from build123d import *

# Parameters (mm, degrees)
SKETCH_1_W                   = 8
SKETCH_1_H                   = 20
EXTRUDE_1_DEPTH              = 10
HOLE_WIZARD_M3_1_D           = 3.4
HOLE_WIZARD_M3_1_CBORE_D     = 6
HOLE_WIZARD_M3_1_CBORE_DEPTH = 6


with BuildPart() as part:
    # 草图1 → 凸台-拉伸1 (new body)
    with BuildSketch(Plane.XY):
        Rectangle(SKETCH_1_W, SKETCH_1_H)
    extrude(amount=EXTRUDE_1_DEPTH)

    # M3 六角圆柱头螺钉的柱形沉头孔1 (through all)
    with Locations(Plane(origin=(4, 0, 0), x_dir=(0, 0, -1), z_dir=(1, 0, 0))):
        with Locations((-5, 5.5), (-5, -5.5)):
            CounterBoreHole(HOLE_WIZARD_M3_1_D / 2, HOLE_WIZARD_M3_1_CBORE_D / 2, HOLE_WIZARD_M3_1_CBORE_DEPTH)

    # 草图4 → 切除-旋转1 (revolve, cut)
    with BuildSketch(Plane(origin=(0, 0, 0), x_dir=(1, 0, 0), z_dir=(0, 1, 0))):
        Polygon((11.5, 1.5), (0.5, 1.5), (1.200682375, -13.581690109), (11.5, -13.581690109), align=None)
    revolve(axis=Axis((11.5, 0, 13.581690109), (0, 0, -1)), mode=Mode.SUBTRACT)


solid = part.part
Work out the finished part from the listing and answer in its coordinate system (mm). A direction names the side the tool comes from. Give positions to 0.01 mm unless a question says otherwise; leave off trailing zeros. Write each loop counter-clockwise with the first axis right and the second up, starting at its lowest first coordinate (ties: lowest second). Pieces come first, ordered by that corner, then holes. Notation, with made-up numbers: (64.5, -4) - (83.5, -4) arc R24 cw to (83.5, 35) - close; hole circle Ø4 at (32.25, 17.5). An arc over 180 degrees is marked (long way). One line per item, written item: value. Start each with the question number.
1. For a pull along Y with two mould halves and no side action, classify faces 3 (the flat face through (4, 9, 5)), 4 (the flat face through (0, 10, 5)), 5 (the flat face through (-2, -7.5, 5)) as +Y half, -Y half, draft (parallel to the pull), parting line (faces both ways), or undercut.
2. Consider probe 1 along Y at (x, z) = (-0.5, 5); probe 2 along Y at (x, z) = (1.5, 5); probe 3 along Y at (x, z) = (-1, 3.75). Determine where each line is inside the solid, lowest interval first.
3. Find section D-D (x = -2.75). Write down the section's boundary in (y, z), then the cut area to 3 significant figures.
4. Find section A-A (x = -1). Write down the section's boundary in (y, z), then the cut area to 3 significant figures.
5. Find section B-B (z = 5). Write down the section's boundary in (x, y).
6. For faces 1 (the flat face through (4, -9, 5)), 2 (the cylindrical face through (0.375, 8.474, 5.391)), determine the directions among +Z, -Z, +X, -X, +Y, -Y from which every point of the face is accessible in a straight line to the end or side of a thin tool.
7. Find section C-C (z = 7). Write down the section's boundary in (x, y).
8. Given pin 1 (1.8 mm diameter, centred on y = -6, z = 6, fed in from +X); pin 2 (2.5 mm diameter, centred on y = 5.5, z = 5, fed in from -X), each flat-ended and moving along its own axis, determine where each tip first touches the part or whether it passes through.
Geometry results:
1. face 3: draft
1. face 4: +Y half
1. face 5: undercut
2. probe 1: -10 to -8.5, -2.5 to 2.5, 8.5 to 10
2. probe 2: -10 to -8.5, 8.5 to 10
2. probe 3: -10 to -8.23, -2.77 to 2.77, 8.23 to 10
3. outline: (-10, 0) - (10, 0) - (10, 10) - (-10, 10) - close; hole circle Ø3.4 at (-5.5, 5); hole circle Ø3.4 at (5.5, 5)
3. area: 182 mm2
4. outline: (-10, 0) - (10, 0) - (10, 10) - (-10, 10) - close; hole circle Ø6 at (-5.5, 5); hole circle Ø6 at (5.5, 5)
4. area: 143 mm2
5. outline: (-4, -10) - (4, -10) - (4, -8.5) - (-2, -8.5) - (-2, -7.2) - (-4, -7.2) - close; (-4, -3.8) - (-2, -3.8) - (-2, -2.5) - (1.1, -2.5) arc R10.7 cw to (1.1, 2.5) - (-2, 2.5) - (-2, 3.8) - (-4, 3.8) - close; (-4, 7.2) - (-2, 7.2) - (-2, 8.5) - (4, 8.5) - (4, 10) - (-4, 10) - close
6. face 1: +Z, -Z, +X, +Y, -Y
6. face 2: +X
7. outline: (-4, -10) - (4, -10) - (4, -7.74) - (-2, -7.74) - (-2, -3.26) - (1.41, -3.26) arc R10.61 cw to (1.41, 3.26) - (-2, 3.26) - (-2, 7.74) - (4, 7.74) - (4, 10) - (-4, 10) - close
8. pin 1: x = -2
8. pin 2: through
